from build123d import *

# Parameters (mm, degrees)
EXTRUDE_1_DEPTH             = 130
SKETCH_2_W                  = 140
SKETCH_2_H                  = 5
CUT_EXTRUDE_1_DEPTH         = 323.645316098
SKETCH_3_W                  = 102
SKETCH_3_H                  = 170
CUT_EXTRUDE_2_DEPTH         = 124
CUT_EXTRUDE_3_DEPTH         = 323.645316098
HOLE_WIZARD_M14_1_D         = 12
HOLE_WIZARD_M14_1_DEPTH     = 34
HOLE_WIZARD_M14_1_TIP       = 3.605163714
HOLE_WIZARD_12_0_12_1_D     = 12
HOLE_WIZARD_12_0_12_1_DEPTH = 34
HOLE_WIZARD_12_0_12_1_TIP   = 3.605163714
CUT_EXTRUDE_4_REACH         = 302.299
SKETCH_12_R                 = 22.5


with BuildPart() as part:
    # 草图1 → 凸台-拉伸1 (new body)
    with BuildSketch(Plane.XY):
        Polygon((0, 0), (-140, 0), (-140, 90), (-50, 260), (0, 260), align=None)
    extrude(amount=EXTRUDE_1_DEPTH)

    # 草图2 → 切除-拉伸1 (cut, through all)
    with BuildSketch(Plane.XY.offset(130)):
        with Locations((-70, 2.5)):
            Rectangle(SKETCH_2_W, SKETCH_2_H)
    extrude(amount=-CUT_EXTRUDE_1_DEPTH, mode=Mode.SUBTRACT)

    # 草图3 → 切除-拉伸2 (cut)
    with BuildSketch(Plane(origin=(-140, 34.772640959, 0), x_dir=(0, 0, -1), z_dir=(1, 0, 0))):
        with Locations((-65, 140.227359041)):
            Rectangle(SKETCH_3_W, SKETCH_3_H)
    extrude(amount=CUT_EXTRUDE_2_DEPTH, mode=Mode.SUBTRACT)

    # 草图5 → 切除-拉伸3 (cut, through all)
    with BuildSketch(Plane.XY.offset(130)):
        Polygon((0, 5), (0, 20), (-15, 5), align=None)
    extrude(amount=-CUT_EXTRUDE_3_DEPTH, mode=Mode.SUBTRACT)

    # M14 螺纹孔1
    with Locations(Plane(origin=(0, 0, 0), x_dir=(0, 0, -1), z_dir=(1, 0, 0))):
        with Locations((-100, 235), (-30, 235), (-100, 115), (-30, 115)):
            Hole(HOLE_WIZARD_M14_1_D / 2, depth=HOLE_WIZARD_M14_1_DEPTH)
            with Locations((0, 0, -(HOLE_WIZARD_M14_1_DEPTH + HOLE_WIZARD_M14_1_TIP / 2))):  # 118° drill point
                Cone(0, HOLE_WIZARD_M14_1_D / 2, HOLE_WIZARD_M14_1_TIP, mode=Mode.SUBTRACT)

    # Ø12.0 (12) 直径孔1
    with Locations(Plane(origin=(0, 0, 0), x_dir=(0, 0, -1), z_dir=(1, 0, 0))):
        with Locations((-105, 175), (-25, 175)):
            Hole(HOLE_WIZARD_12_0_12_1_D / 2, depth=HOLE_WIZARD_12_0_12_1_DEPTH)
            with Locations((0, 0, -(HOLE_WIZARD_12_0_12_1_DEPTH + HOLE_WIZARD_12_0_12_1_TIP / 2))):  # 118° drill point
                Cone(0, HOLE_WIZARD_12_0_12_1_D / 2, HOLE_WIZARD_12_0_12_1_TIP, mode=Mode.SUBTRACT)

    # 草图12 → 切除-拉伸4 (cut, up to next)
    with BuildSketch(Plane(origin=(-90.854033512, 5, 0), x_dir=(-1, 0, 0), z_dir=(0, 1, 0)), mode=Mode.PRIVATE) as cut_extrude_4_sk1:
        with Locations(Location((-0.854033512, 63, 0), (0, 0, 90))):
            Circle(SKETCH_12_R)
    cut_extrude_4_tool1 = extrude(cut_extrude_4_sk1.sketch, amount=CUT_EXTRUDE_4_REACH, mode=Mode.PRIVATE) & part.part
    add(cut_extrude_4_tool1.solids().sort_by_distance((-90, 5, 63))[0], mode=Mode.SUBTRACT)


solid = part.part
For this review, take the finished solid that the model builds, in its own axes (mm). A direction names the side the tool comes from. Give positions to 0.01 mm unless a question says otherwise; leave off trailing zeros. Order: outer loops, then holes, each group sorted by start corner. A loop starts at its lowest first (then second) coordinate and runs counter-clockwise, first axis right, second up. Notation, with made-up numbers: M 82,63 L 116,63 A25 cw 116,86 Z; hole C 70.25,82.5 d8. An arc over 180 degrees is marked long. Answer in a Markdown table with one row per item. Add a question column.
(1) For faces 1 (the face through (-65, 90, 66)), 2 (the face through (-8.112, 169.143, 23.699)), list the 3-axis set-ups (+Z, -Z, +X, -X, +Y, -Y) from which the entire face can be reached by the end or side of a thin tool; tool diameter is ignored.
(2) Consider section A-A on y = 175. State the section outline as (x, z) points, and give its area (3 significant figures).
(3) Consider section C-C on z = 46.5. State the section outline as (x, y) points.
(4) For pin 1 (6 mm diameter, centred on y = 141.5, z = 76.5, fed in from +X); pin 2 (3 mm diameter, centred on x = -28, z = 110, fed in from +Y); pin 3 (2 mm diameter, centred on y = 118, z = 87, fed in from -X); pin 4 (11 mm diameter, centred on y = 235, z = 100, fed in from +X) (3 decimals), all flat-tipped, find the tip position at first contact; note any pin that passes through.
(5) Consider section B-B on x = -9.5. State the section outline as (y, z) points, and give its area (3 significant figures).
(6) Wall thickness on probe 1 along Y at (x, z) = (-12, 100); probe 2 along Y at (x, z) = (-11.5, 25); probe 3 along Z at (x, y) = (-60.5, 188.5): over which ranges is each line inside the solid? List them lowest first. Write a range as [from, to].
(7) Mouldability with a two-part tool opening along Y and no side actions: class faces 3 (the face through (-14, 260, 64)), 4 (the face through (-74.79, 46.9, 46.42)), 5 (the face through (-7, 13, 66)), 6 (the face through (-8.11, 239.06, 95.58)) as +Y half, -Y half, draft (parallel to the pull), parting line (faces both ways), or undercut.
(8) Consider section D-D on y = 31. State the section outline as (x, z) points.
Evaluation:
| question | item | result |
|---|---|---|
| 1 | face 1 | -X, +Y |
| 1 | face 2 | +X, -X |
| 2 | outline | M -95,0 L 0,0 L 0,19 L -16,19 L -16,14 L -95,14 Z; M -95,116 L -16,116 L -16,111 L 0,111 L 0,130 L -95,130 Z; M -16,31 L 0,31 L 0,99 L -16,99 Z |
| 2 | area | 3,910 mm^2 |
| 3 | outline | M -140,5 L -105.3,5 L -105.3,90 L -140,90 Z; M -74.7,5 L -15,5 L 0,20 L 0,260 L -16,260 L -16,90 L -74.7,90 Z |
| 4 | pin 1 | stops at x = 0 |
| 4 | pin 2 | stops at y = 90 |
| 4 | pin 3 | stops at x = -16 |
| 4 | pin 4 | passes through |
| 5 | outline | M 10.5,0 L 260,0 L 260,130 L 10.5,130 Z; hole C 115,30 d12; hole C 115,100 d12; hole C 175,25 d12; hole C 175,105 d12; hole C 235,30 d12; hole C 235,100 d12 |
| 5 | area | 31,800 mm^2 |
| 6 | probe 1 | y = [8, 109], [121, 171.68], [178.32, 229], [241, 260] |
| 6 | probe 2 | y = [8.5, 111.68], [118.32, 169], [181, 231.68], [238.32, 260] |
| 6 | probe 3 | z = [0, 14], [116, 130] |
| 7 | face 3 | +Y half |
| 7 | face 4 | draft |
| 7 | face 5 | -Y half |
| 7 | face 6 | undercut |
| 8 | outline | M -140,0 L 0,0 L 0,130 L -140,130 Z; hole C -90,63 d45 |
